Read the model definition and answer for the solid it produces. Units are mm, in the model's axes. Face numbers are marked on the shaded views. A direction names the side the tool comes from. Round coordinates to 2 decimals unless told otherwise and drop trailing zeros. Order: outer loops, then holes, each group sorted by start corner. A loop starts at its lowest first (then second) coordinate and runs counter-clockwise, first axis right, second up. Notation, with made-up numbers: (48, 66.25) - (81, 66.25) arc R25 cw to (81, 105.25) - close; hole circle Ø2 at (-4, -13). An arc over 180 degrees is marked (long way). Put each result on its own line as item: value. Start each with the question number.
Q1. Which of the six approach directions +Z, -Z, +X, -X, +Y, -Y give full straight-line access (tool end or side, diameter ignored) to the marked faces 5, 6 and 7?
Q2. Each of these flat-tipped pins is pushed along its axis until it touches: pin 1 Ø2 at (x, z) = (101, 21) entering from -Y; pin 2 Ø6 at (y, z) = (-64.5, -40) entering from -X; pin 3 Ø5 at (x, y) = (70, -2.5) entering from -Z. Where does it stop, or does it pass through?
Q3. For a pull along Z with two mould halves and no side action, classify the marked faces 1, 2, 3 and 4 as pulls with the +Z half, pulls with the -Z half, needs draft (parallel to the pull), parting line crosses it, or undercut.
Q4. Section B-B on z = -45 is taken. State how many separate pieces and enclosed holes the cut face has, then the cut area to 3 significant figures.
Q5. Section A-A on x = 57 is taken. Give the vertices of the cut face in (y, z).
Q6. Find the intervals of material crossed by line 1 along Y through (x, z) = (12.5, 0); line 2 along X through (y, z) = (44.5, 69.5); line 3 along X through (y, z) = (71, -12), in increasing order. Write a range as from..to.
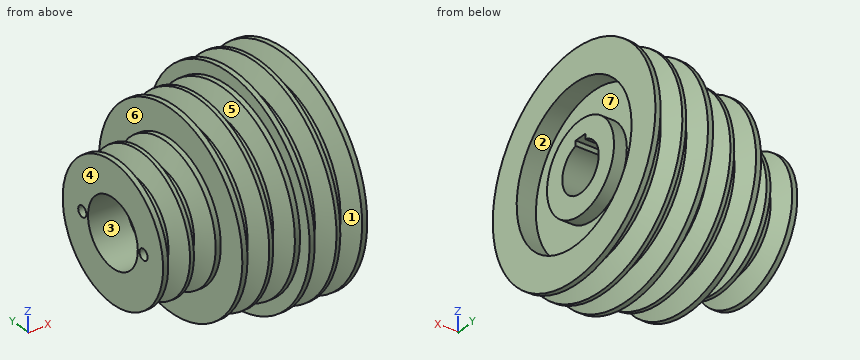
from build123d import *

# Parameters (mm, degrees)
HOLE_WIZARD_M10_1_D     = 8.5
HOLE_WIZARD_M10_1_DEPTH = 24.5
HOLE_WIZARD_M10_1_TIP   = 2.553657631
SKETCH_6_W              = 3.96969722
SKETCH_6_H              = 10
CUT_EXTRUDE_1_DEPTH     = 178.059312096


with BuildPart() as part:
    # 草图1 → 旋转1 (revolve)
    with BuildSketch(Plane.XY, mode=Mode.PRIVATE) as revolve_1_sk:
        Polygon((0, 26), (0, 52.5), (4, 52.5), (8.891690903, 36.5), (16.108309097, 36.5), (21, 52.5), (24, 52.5), (28.891690903, 36.5), (36.108309097, 36.5), (41, 52.5), (45, 52.5), (45, 75), (49, 75), (53.891690903, 59), (61.108309097, 59), (66, 75), (69, 75), (73.891690903, 59), (81.108309097, 59), (86, 75), (90, 75), (90, 85), (94, 85), (98.891690903, 69), (106.108309097, 69), (111, 85), (114, 85), (118.891690903, 69), (126.108309097, 69), (131, 85), (135, 85), (135, 60), (120, 60), (120, 35), (130, 35), (130, 19), (30, 19), (30, 26), align=None)
    revolve(revolve_1_sk.sketch.rotate(Axis((-46.234880066, 0, 0), (1, 0, 0)), 90), axis=Axis((-46.234880066, 0, 0), (1, 0, 0)))

    # M10 螺纹孔1
    with Locations(Plane.ZY):
        with Locations((0, 32), (0, -32)):
            Hole(HOLE_WIZARD_M10_1_D / 2, depth=HOLE_WIZARD_M10_1_DEPTH)
            with Locations((0, 0, -(HOLE_WIZARD_M10_1_DEPTH + HOLE_WIZARD_M10_1_TIP / 2))):  # 118° drill point
                Cone(0, HOLE_WIZARD_M10_1_D / 2, HOLE_WIZARD_M10_1_TIP, mode=Mode.SUBTRACT)

    # 草图6 → 切除-拉伸1 (cut, through all)
    with BuildSketch(Plane(origin=(130, 0, 0), x_dir=(0, 0, -1), z_dir=(1, 0, 0))):
        with Locations((-20.31515139, 0)):
            Rectangle(SKETCH_6_W, SKETCH_6_H)
    extrude(amount=-CUT_EXTRUDE_1_DEPTH, mode=Mode.SUBTRACT)


solid = part.part
Findings:
1. face 5: none
1. face 6: -X
1. face 7: +X
2. pin 1: y = -66.04
2. pin 2: x = 45
2. pin 3: z = -75
3. face 1: parting line crosses it
3. face 2: undercut
3. face 3: undercut
3. face 4: needs draft
4. separate pieces: 3
4. enclosed holes: 0
4. area: 9,620 mm2
5. outline: circle Ø118 at (0, 0); hole (-5, 18.33) arc R19 ccw (long way) to (5, 18.33) - (5, 22.3) - (-5, 22.3) - close
6. line 1: -36.5..-36.25, -27.75..-26, 26..27.75, 36.25..36.5
6. line 2: 90..94.76, 110.24..114.76, 130.24..135
6. line 3: 45..49.92, 65.08..69.92, 85.08..97.97, 107.03..117.97, 127.03..135
